```python
from build123d import *


with BuildPart() as part:
    # Sketch1 → Revolve1 (revolve)
    with BuildSketch(Plane.XY):
        Polygon((-29.5, 0), (-58, 0), (-60, 2), (-60, 16), (-55, 21), (-40, 21), (-40, 44), (-38, 46), (-29.5, 46), (-27.5, 44), (-27.5, 2), align=None)
    revolve(axis=Axis((0, 46, 0), (0, -1, 0)))


solid = part.part
```
Work out the finished part from the listing and answer in its coordinate system (mm). A direction names the side the tool comes from. Give positions to 0.01 mm unless a question says otherwise; leave off trailing zeros. Order: outer loops, then holes, each group sorted by start corner. A loop starts at its lowest first (then second) coordinate and runs counter-clockwise, first axis right, second up.
1. Straight lines are drawn through the part: L1, parallel to X at y = 24, z = 0; L2, parallel to Z at x = 0, y = 13. For each, find the intervals that lie inside material, in ascending order.
Result sheet:
L1: x = -40 to -27.5, 27.5 to 40
L2: z = -60 to -27.5, 27.5 to 60
2. Section D-D, the plane y = 18.5 is taken. Determine the outline of the cut face in (x, z), and give its area (3 significant figures).
Result sheet:
outline: circle Ø115 at (0, 0); hole circle Ø55 at (0, 0)
area: 8,010 mm2
3. Section A-A, the plane x = 0 is taken. Determine the outline of the cut face in (y, z).
Result sheet:
outline: (0, -58) - (2, -60) - (16, -60) - (21, -55) - (21, -40) - (44, -40) - (46, -38) - (46, -29.5) - (44, -27.5) - (2, -27.5) - (0, -29.5) - close; (0, 29.5) - (2, 27.5) - (44, 27.5) - (46, 29.5) - (46, 38) - (44, 40) - (21, 40) - (21, 55) - (16, 60) - (2, 60) - (0, 58) - close
4. Each of these flat-tipped pins is pushed along its axis until it touches: P1, Ø3, axis at y = 27, z = 6.5, coming from the -X side; P2, Ø2, axis at y = 5, z = 10.5, coming from the -X side; P3, Ø12, axis at y = 35.5, z = -37, coming from the -X side. Where does it stop, or does it pass through?
Result sheet:
P1: stops at x = -39.69
P2: stops at x = -59.24
P3: stops at x = -25.28
5. The mould has two halves that part along X. Classify faces 1 (the cylindrical face through (5.961, 22.706, 26.846)), 2 (the flat face through (-20, 46, 22)), 3 (the conical face through (-12.75, 1.87, 24.51)), 4 (the cylindrical face through (59.94, 9.1, -2.64)): released by +X, released by -X, zero draft, split by the parting line, or undercut.
Result sheet:
face 1: undercut
face 2: zero draft
face 3: undercut
face 4: split by the parting line
6. Section C-C, the plane y = 28 is taken. Determine the outline of the cut face in (x, z).
Result sheet:
outline: circle Ø80 at (0, 0); hole circle Ø55 at (0, 0)
7. Section B-B, the plane z = 0 is taken. Determine the outline of the cut face in (x, y), and give its area (3 significant figures).
Result sheet:
outline: (-60, 2) - (-58, 0) - (-29.5, 0) - (-27.5, 2) - (-27.5, 44) - (-29.5, 46) - (-38, 46) - (-40, 44) - (-40, 21) - (-55, 21) - (-60, 16) - close; (27.5, 2) - (29.5, 0) - (58, 0) - (60, 2) - (60, 16) - (55, 21) - (40, 21) - (40, 44) - (38, 46) - (29.5, 46) - (27.5, 44) - close
area: 1,950 mm2
8. For faces 5 (the conical face through (7.567, 0.125, -57.63)), 6 (the cylindrical face through (8.67, 32.66, 39.05)), determine the directions among +Z, -Z, +X, -X, +Y, -Y from which every point of the face is accessible in a straight line to the end or side of a thin tool.
Result sheet:
face 5: -Y
face 6: +Y
